CAD build for the part. Positions are in the model's coordinates, mm. A direction names the side the tool comes from. Coordinates: 2 decimals unless noted, no trailing zeros. Order: outer loops, then holes, each group sorted by start corner. A loop starts at its lowest first (then second) coordinate and runs counter-clockwise, first axis right, second up. Notation, with made-up numbers: (32, -35) - (60, -35) arc R24 cw to (60, -7) - close; hole circle Ø9 at (6, -2.75). An arc over 180 degrees is marked (long way). Return JSON: item names as keys, results as strings.
from build123d import *

# Parameters (mm, degrees)
SKETCH_1_R          = 8.5
EXTRUDE_1_DEPTH     = 5
FILLET_1_R          = 2
CUT_EXTRUDE_1_REACH = 57.057
SKETCH_2_R          = 2.75


with BuildPart() as part:
    # 草图1 → 凸台-拉伸1 (new, symmetric)
    with BuildSketch(Plane.XY):
        Polygon((0, 0), (-22.5, 0), (-22.5, 7), (-12.5, 7), (-12.5, 57), (12.5, 57), (12.5, 7), (22.5, 7), (22.5, 0), align=None)
        with Locations((0, 45)):
            Circle(SKETCH_1_R, mode=Mode.SUBTRACT)
    extrude(amount=EXTRUDE_1_DEPTH, both=True)

    # 圆角1
    fillet_1_edges = [part.edges().sort_by_distance(p)[0] for p in [
        (-12.5, 57, 0),
        (12.5, 57, 0),
    ]]
    fillet(fillet_1_edges, radius=FILLET_1_R)

    # 草图2 → 切除-拉伸1 (cut, up to next)
    with BuildSketch(Plane(origin=(0, 7, 0), x_dir=(1, 0, 0), z_dir=(0, 1, 0)), mode=Mode.PRIVATE) as cut_extrude_1_sk1:
        with Locations(Location((-17.5, 0, 0), (0, 0, 180))):
            Circle(SKETCH_2_R)
    cut_extrude_1_tool1 = extrude(cut_extrude_1_sk1.sketch, amount=-CUT_EXTRUDE_1_REACH, mode=Mode.PRIVATE) & part.part
    # 草图2 → 切除-拉伸1 (cut, up to next)
    with BuildSketch(Plane(origin=(0, 7, 0), x_dir=(1, 0, 0), z_dir=(0, 1, 0)), mode=Mode.PRIVATE) as cut_extrude_1_sk2:
        with Locations(Location((17.5, 0, 0), (0, 0, 180))):
            Circle(SKETCH_2_R)
    cut_extrude_1_tool2 = extrude(cut_extrude_1_sk2.sketch, amount=-CUT_EXTRUDE_1_REACH, mode=Mode.PRIVATE) & part.part
    add(cut_extrude_1_tool1.solids().sort_by_distance((-17.5, 7, 0))[0], mode=Mode.SUBTRACT)
    add(cut_extrude_1_tool2.solids().sort_by_distance((17.5, 7, 0))[0], mode=Mode.SUBTRACT)


solid = part.part
Item 1: Mould opens along Z. For faces 1 (the flat face through (-12.5, 31, 0)), 2 (the cylindrical face through (20.247, 3.549, 0.121)), 3 (the flat face through (0, 23, 5)) say: released by +Z, released by -Z, zero draft, split by the parting line, or undercut.
Findings below:
{"face 1": "zero draft", "face 2": "undercut", "face 3": "released by +Z"}
Item 2: Band-saw the part on B-B, the plane z = 0. List the corners of the cut face in (x, y).
Findings below:
{"outline": "(-22.5, 0) - (-20.25, 0) - (-20.25, 7) - (-22.5, 7) - close; (-14.75, 0) - (14.75, 0) - (14.75, 7) - (12.5, 7) - (12.5, 55) arc R2 ccw to (10.5, 57) - (-10.5, 57) arc R2 ccw to (-12.5, 55) - (-12.5, 7) - (-14.75, 7) - close; (20.25, 0) - (22.5, 0) - (22.5, 7) - (20.25, 7) - close; hole circle Ø17 at (0, 45)"}
Item 3: Band-saw the part on A-A, the plane y = 49. List the corners of the cut face in (x, z).
Findings below:
{"outline": "(-12.5, -5) - (-7.5, -5) - (-7.5, 5) - (-12.5, 5) - close; (7.5, -5) - (12.5, -5) - (12.5, 5) - (7.5, 5) - close"}
Item 4: Drop flat-ended pins along their axis: P1, Ø3, axis at x = -17.5, z = 1.5, coming from the +Y side; P2, Ø6, axis at y = 42.5, z = -2.5, coming from the -X side; P3, Ø5, axis at x = 17.5, z = 0, coming from the -Y side; P4, Ø5, axis at y = 30, z = -2.5, coming from the +X side. Give the stop position or say it passes through.
Findings below:
{"P1": "stops at y = 7", "P2": "stops at x = -12.5", "P3": "passes through", "P4": "stops at x = 12.5"}
Item 5: Band-saw the part on C-C, the plane x = -17.5. List the corners of the cut face in (y, z), then the cut area to 3 significant figures.
Findings below:
{"outline": "(0, -5) - (7, -5) - (7, -2.75) - (0, -2.75) - close; (0, 2.75) - (7, 2.75) - (7, 5) - (0, 5) - close", "area": "31.5 mm²"}
Item 6: Band-saw the part on D-D, the plane y = 8. List the corners of the cut face in (x, z), then the cut area to 3 significant figures.
Findings below:
{"outline": "(-12.5, -5) - (12.5, -5) - (12.5, 5) - (-12.5, 5) - close", "area": "250 mm²"}
Item 7: Which spindle directions (+Z, -Z, +X, -X, +Y, -Y) get a long thin tool onto all of the face, cutting with end or side? Do faces 4 (the flat face through (15, 7, -2)), 5 (the flat face through (0, 57, 0)), 6 (the flat face through (-20, 7, -2)). Say none if no direction does.
Findings below:
{"face 4": "+Z, -Z, +X, +Y", "face 5": "+Z, -Z, +X, -X, +Y", "face 6": "+Z, -Z, -X, +Y"}
Item 8: Wall check: L1, parallel to Y at x = 0, z = -0.5; L2, parallel to X at y = 44.5, z = -2; L3, parallel to Z at x = -17.5, y = 1.5. Give the ranges that are in metal, low to high. Write a range as [from, to].
Findings below:
{"L1": "y = [0, 36.5], [53.5, 57]", "L2": "x = [-12.5, -8.49], [8.49, 12.5]", "L3": "z = [-5, -2.75], [2.75, 5]"}
